from build123d import *

# Parameters (mm, degrees)
SKETCH1_R           = 25
SKETCH1_R_2         = 15
BOSS_EXTRUDE1_DEPTH = 60
CHAMFER1_SIZE       = 1


with BuildPart() as part:
    # Sketch1 → Boss-Extrude1 (new body)
    with BuildSketch(Plane.XY):
        Circle(SKETCH1_R)
        Circle(SKETCH1_R_2, mode=Mode.SUBTRACT)
    extrude(amount=BOSS_EXTRUDE1_DEPTH)

    # Chamfer1
    chamfer1_edges = [part.edges().sort_by_distance(p)[0] for p in [
        (-25, 0, 0),
        (-25, 0, 60),
        (-15, 0, 0),
        (-15, 0, 60),
    ]]
    chamfer(chamfer1_edges, length=CHAMFER1_SIZE)


solid = part.part
Build history of the part. All positions in model axes, mm. Coordinates: 2 decimals unless noted, no trailing zeros. Order: outer loops, then holes, each group sorted by start corner. A loop starts at its lowest first (then second) coordinate and runs counter-clockwise, first axis right, second up. Notation, with made-up numbers: (0.25, 16.5) - (20.25, 16.5) arc R14 ccw to (20.25, 24.5) - close; hole circle Ø2 at (-14.5, 62). An arc over 180 degrees is marked (long way). Write item = value, one per line. Start each with the question number.
1) Saw through at C-C on z = 52. Write the cut outline in (x, y).
2) Flat gauge pins, fed straight in: pin 1 Ø4 at (x, y) = (10.5, 9.5) entering from -Z; pin 2 Ø1.5 at (x, z) = (2.5, 7.5) entering from -Y; pin 3 Ø1.5 at (y, z) = (8.5, 16.5) entering from -X; pin 4 Ø1 at (y, z) = (-19, 19) entering from +X. Where does each tip first touch, or does it go through?
3) Saw through at A-A on y = 0. Write the cut outline in (x, z).
4) Wall check: line 1 along Y through (x, z) = (0, 21); line 2 along Y through (x, z) = (-2, 42.5); line 3 along X through (y, z) = (7.5, 8.5). Give the ranges that are in metal, low to high. Write a range as from..to.
5) Two-plate mould, pull along X, no slides. Class faces 1 (the face through (-14.985, 0.66, 29.594)), 2 (the face through (23.846, 7.509, 29.594)), 3 (the face through (5, -16, 0)): pulls with the +X half, pulls with the -X half, needs draft (parallel to the pull), parting line crosses it, or undercut.
From the geometry:
q1.outline = circle Ø50 at (0, 0); hole circle Ø30 at (0, 0)
q2.pin_1 = 0
q2.pin_2 = -24.94
q2.pin_3 = -23.77
q2.pin_4 = 16.82
q3.outline = (-25, 1) - (-24, 0) - (-16, 0) - (-15, 1) - (-15, 59) - (-16, 60) - (-24, 60) - (-25, 59) - close; (15, 1) - (16, 0) - (24, 0) - (25, 1) - (25, 59) - (24, 60) - (16, 60) - (15, 59) - close
q4.line_1 = -25..-15, 15..25
q4.line_2 = -24.92..-14.87, 14.87..24.92
q4.line_3 = -23.85..-12.99, 12.99..23.85
q5.face_1 = undercut
q5.face_2 = parting line crosses it
q5.face_3 = needs draft
